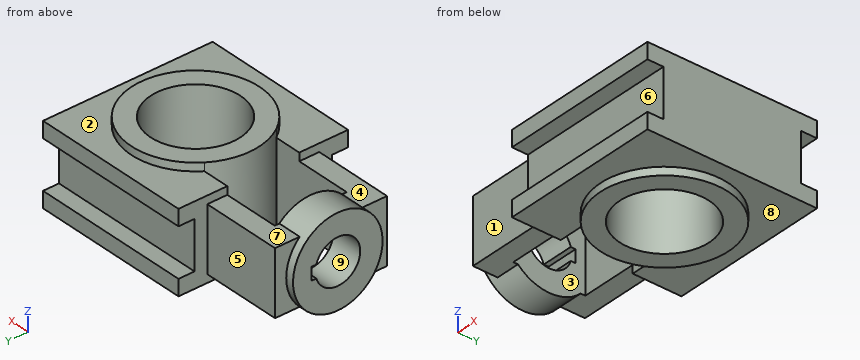
```python
from build123d import *

# Parameters (mm, degrees)
BASE_BLOCK_PROFILE_W         = 100
BASE_BLOCK_PROFILE_H         = 106
BASE_BLOCK_DEPTH             = 25
HOUSING_BOSS_PROFILE_W       = 50
HOUSING_BOSS_PROFILE_H       = 70
HOUSING_BOSS_DEPTH           = 20
GUIDE_KEY_SLOTS_PROFILE_W    = 30
GUIDE_KEY_SLOTS_PROFILE_H    = 10
GUIDE_KEY_SLOTS_DEPTH        = 100
BEARING_BOSS_PROFILE_80_R    = 40
BEARING_BOSS_80_DEPTH        = 30
BEARING_COLLAR_56_DEPTH      = 5
BEARING_COLLAR_56_DEPTH_BACK = 15
BEARING_COLLAR_PROFILE_56_R  = 28
BEARING_BORE_DEPTH           = 122.383689184
BEARING_BORE_DEPTH_BACK      = 122.383689184
BEARING_BORE_PROFILE_R       = 28
BORE_KEYWAY_DEPTH            = 20


with BuildPart() as part:
    # Base Block Profile → Base Block (new, symmetric)
    with BuildSketch(Plane.XY):
        Rectangle(BASE_BLOCK_PROFILE_W, BASE_BLOCK_PROFILE_H)
    extrude(amount=BASE_BLOCK_DEPTH, both=True)

    # Housing Boss Profile → Housing Boss (add, symmetric)
    with BuildSketch(Plane.XY):
        with Locations((-75, 0)):
            Rectangle(HOUSING_BOSS_PROFILE_W, HOUSING_BOSS_PROFILE_H)
    extrude(amount=HOUSING_BOSS_DEPTH, both=True)

    # Guide Key Slots Profile → Guide Key Slots (cut)
    with BuildSketch(Plane.ZY.offset(50)):
        with Locations((0, 48)):
            Rectangle(GUIDE_KEY_SLOTS_PROFILE_W, GUIDE_KEY_SLOTS_PROFILE_H)
        with Locations((0, -48)):
            Rectangle(GUIDE_KEY_SLOTS_PROFILE_W, GUIDE_KEY_SLOTS_PROFILE_H)
    extrude(amount=-GUIDE_KEY_SLOTS_DEPTH, mode=Mode.SUBTRACT)

    # Bearing Boss Profile Ø80 → Bearing Boss Ø80 (add, symmetric)
    with BuildSketch(Plane.XY):
        with Locations(Location((0, 0, 0), (0, 0, 180))):
            Circle(BEARING_BOSS_PROFILE_80_R)
    extrude(amount=BEARING_BOSS_80_DEPTH, both=True)

    # Bearing Collar Profile Ø56 → Bearing Collar Ø56 (add, two sides: drawn at the far end of the back side and taken through both)
    with BuildSketch(Plane.ZY.offset(100).offset(-BEARING_COLLAR_56_DEPTH_BACK)):
        with Locations(Location((0, 0, 0), (0, 0, 224.415308597))):
            Circle(BEARING_COLLAR_PROFILE_56_R)
    extrude(amount=BEARING_COLLAR_56_DEPTH + BEARING_COLLAR_56_DEPTH_BACK)

    # Bearing Bore Profile → Bearing Bore (cut, two sides: drawn at the far end of the back side and taken through both)
    with BuildSketch(Plane.XY.offset(-BEARING_BORE_DEPTH_BACK)):
        Circle(BEARING_BORE_PROFILE_R)
        with BuildLine():
            Line((-85, 22.5), (-33.071891388, 22.5))
            ThreePointArc((-33.071891388, 22.5), (-40, 0), (-33.071891388, -22.5))
            Line((-33.071891388, -22.5), (-85, -22.5))
            Line((-85, -22.5), (-85, 22.5))
        make_face()
    extrude(amount=BEARING_BORE_DEPTH + BEARING_BORE_DEPTH_BACK, mode=Mode.SUBTRACT)

    # Bore Keyway Profile → Bore Keyway (cut)
    with BuildSketch(Plane.ZY.offset(105)):
        with BuildLine():
            Line((-4, 13.416407865), (-4, 16.416407865))
            Line((-4, 16.416407865), (4, 16.416407865))
            Line((4, 16.416407865), (4, 13.416407865))
            ThreePointArc((4, 13.416407865), (0, -14), (-4, 13.416407865))
        make_face()
    extrude(amount=-BORE_KEYWAY_DEPTH, mode=Mode.SUBTRACT)


solid = part.part
```
Check sheet for the modelled part. Datum: model origin and axes. Units: mm. Face numbers are marked on the shaded views. A direction names the side the tool comes from. Coordinates: 2 decimals unless noted, no trailing zeros. Order: outer loops, then holes, each group sorted by start corner. A loop starts at its lowest first (then second) coordinate and runs counter-clockwise, first axis right, second up. Notation, with made-up numbers: (88.25, 28) -> (141.25, 28) arc R15 cw to (141.25, 47) -> close; hole circle Ø3 at (87.25, 43). An arc over 180 degrees is marked (long way). Write each question's results on one line, items separated by ' | '. Start each with the question number.
1) Section check D-D (x = 1.5). Enter the section's corners in (y, z).
2) Section check A-A (x = -74.5). Enter the section's corners in (y, z).
3) Section check C-C (z = 0). Enter the section's corners in (x, y).
4) Draft check along Z on the marked faces 6, 7, 8 and 9. Enter one of: pulls with the +Z half, pulls with the -Z half, needs draft (parallel to the pull), parting line crosses it, or undercut.
5) Section check B-B (y = 0). Enter the section's corners in (x, z).
6) Depth check by flat-ended pin: pin 1 (4.5 mm diameter, centred on x = -71.5, y = 26, fed in from -Z); pin 2 (24 mm diameter, centred on x = 11, z = 0, fed in from +Y); pin 3 (3 mm diameter, centred on x = 0, y = -47.5, fed in from +Z). Enter the tip coordinate at first touch or a pass-through.
7) Set-up check for the marked faces 1, 2, 3, 4 and 5: record each of +Z, -Z, +X, -X, +Y, -Y from which the full face is reachable in a straight line by a thin tool's end or side.
8) Material ranges on line 1 along X through (y, z) = (0, 6); line 2 along Y through (x, z) = (-68, 5); line 3 along Z through (x, y) = (-98, 0), recorded low to high.
Checked values:
1) outline: (-53, -25) -> (-39.97, -25) -> (-39.97, -30) -> (-27.96, -30) -> (-27.96, 30) -> (-39.97, 30) -> (-39.97, 25) -> (-53, 25) -> (-53, 15) -> (-43, 15) -> (-43, -15) -> (-53, -15) -> close; (27.96, -30) -> (39.97, -30) -> (39.97, -25) -> (53, -25) -> (53, -15) -> (43, -15) -> (43, 15) -> (53, 15) -> (53, 25) -> (39.97, 25) -> (39.97, 30) -> (27.96, 30) -> close
2) outline: (-35, -20) -> (-22.5, -20) -> (-22.5, 20) -> (-35, 20) -> close; (22.5, -20) -> (35, -20) -> (35, 20) -> (22.5, 20) -> close
3) outline: (-105, -28) -> (-100, -28) -> (-100, -35) -> (-50, -35) -> (-50, -43) -> (50, -43) -> (50, 43) -> (-50, 43) -> (-50, 35) -> (-100, 35) -> (-100, 28) -> (-105, 28) -> (-105, 16.42) -> (-85, 16.42) -> (-85, 22.5) -> (-33.07, 22.5) arc R40 ccw to (-33.07, -22.5) -> (-85, -22.5) -> (-85, -14) -> (-105, -14) -> close; hole circle Ø56 at (0, 0)
4) face 6: undercut | face 7: pulls with the +Z half | face 8: pulls with the -Z half | face 9: undercut
5) outline: (-105, -28) -> (-85, -28) -> (-85, -14) -> (-105, -14) -> close; (-105, 14) -> (-85, 14) -> (-85, 28) -> (-105, 28) -> close; (-40, -30) -> (-28, -30) -> (-28, 30) -> (-40, 30) -> close; (28, -30) -> (40, -30) -> (40, -25) -> (50, -25) -> (50, 25) -> (40, 25) -> (40, 30) -> (28, 30) -> close
6) pin 1: z = -20 | pin 2: y = 43 | pin 3: z = 25
7) face 1: +Z, -Z, -X, -Y | face 2: +Z | face 3: +Z, -Z | face 4: +Z, -X, -Y | face 5: +Z, -Z, -X, +Y
8) line 1: -40 to -28, 28 to 50 | line 2: -35 to -22.5, 22.5 to 35 | line 3: -28 to -14, 14 to 28
